Part model, mm, in its own coordinate system. Face numbers are marked on the shaded views. A direction names the side the tool comes from. Give positions to 0.01 mm unless a question says otherwise; leave off trailing zeros. Order: outer loops, then holes, each group sorted by start corner. A loop starts at its lowest first (then second) coordinate and runs counter-clockwise, first axis right, second up.
1. Probe line 1 (X direction, y = -26, z = -0.75); line 2 (Z direction, x = 0, y = -138.5); line 3 (Z direction, x = 1, y = -236.5). List the from-to ranges inside material, lowest first.
2. Slice it at B-B on x = 46. List the corners of the cut face in (y, z).
3. Which spindle directions (+Z, -Z, +X, -X, +Y, -Y) get a long thin tool onto all of the face, cutting with end or side? Do the marked faces 1 and 2. Say none if no direction does.
4. Drop flat-ended pins along their axis: pin 1 Ø8 at (x, z) = (65.5, -4.5) entering from +Y; pin 2 Ø12 at (y, z) = (-72, 2.5) entering from +X; pin 3 Ø3 at (y, z) = (-189, 6) entering from -X. Give the stop position or say it passes through.
5. Slice it at A-A on z = 0. List the corners of the cut face in (x, y), and give its area (3 significant figures).
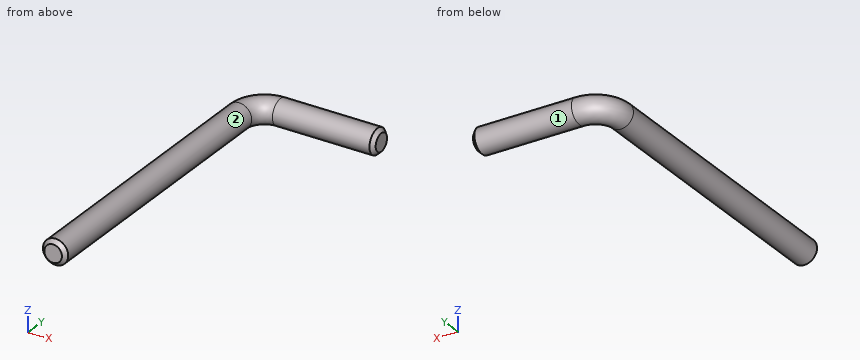
from build123d import *

# Parameters (mm, degrees)
SWEEP_1_PROFILE_R = 10
CHAMFER_1_SIZE    = 3
CHAMFER_2_SIZE    = 3


with BuildPart() as part:
    # 扫描1: sweep along a path in 草图1
    with BuildLine(Plane.XY) as sweep_1_path:
        Line((0, -250), (0, -20))
        ThreePointArc((0, -20), (5.857864376, -5.857864376), (20, 0))
        Line((20, 0), (100, 0))
    # 扫描1 profile (on start of the path) → 扫描1 (sweep)
    with BuildSketch(Plane(origin=(0, -250, 0), x_dir=(1, 0, 0), z_dir=(0, 1, 0))):
        Circle(SWEEP_1_PROFILE_R)
    sweep(path=sweep_1_path.line)

    # 倒角1
    chamfer_1_edges = [part.edges().sort_by_distance(p)[0] for p in [
        (-10, -250, 0),
    ]]
    chamfer(chamfer_1_edges, length=CHAMFER_1_SIZE)

    # 倒角2
    chamfer_2_edges = [part.edges().sort_by_distance(p)[0] for p in [
        (100, 10, 0),
    ]]
    chamfer(chamfer_2_edges, length=CHAMFER_2_SIZE)


solid = part.part
Data:
1. line 1: x = -9.97 to 9.97
1. line 2: z = -10 to 10
1. line 3: z = -9.95 to 9.95
2. outline: circle Ø20 at (0, 0)
3. face 1: +X
3. face 2: -Y
4. pin 1: stops at y = 9.99
4. pin 2: stops at x = 10
4. pin 3: stops at x = -8.93
5. outline: (-10, -247) - (-7, -250) - (7, -250) - (10, -247) - (10, -20) arc R10 cw to (20, -10) - (97, -10) - (100, -7) - (100, 7) - (97, 10) - (20, 10) arc R30 ccw to (-10, -20) - close
5. area: 6,810 mm2
